Can you work these out from the model? Positions are in its coordinate system, mm. Round coordinates to 2 decimals unless told otherwise and drop trailing zeros. Loops run counter-clockwise (first coordinate to the right, second up) from the corner with the lowest first, then second, coordinate; pieces in that order, holes last.
(1) I want a section at A-A on y = 130. Write out the boundary of the cut face in (x, z).
(2) Will these pins go through, and if not, where does the flat tip stop? pin 1 Ø5 at (y, z) = (180.5, -30) entering from -X; pin 2 Ø25 at (y, z) = (527, 10) entering from -X; pin 3 Ø6 at (y, z) = (816, 2.5) entering from +X; pin 4 Ø22.5 at (y, z) = (50, -0.08) entering from -X.
(3) I want a section at C-C on y = 481.5. Write out the boundary of the cut face in (x, z).
(4) If I drill on line 1 along Z through (x, y) = (3, 1070); line 2 along Z through (x, y) = (15, 241); line 3 along Y through (x, z) = (-6, 7.5), over which ranges is the centre line in solid material (lowest first)?
(5) I want a section at B-B on z = -2.5. Write out the boundary of the cut face in (x, y), plus the area to 3 significant figures.
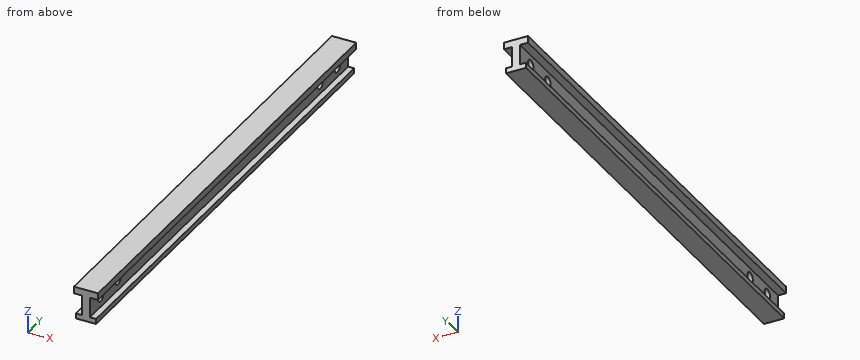
from build123d import *

# Parameters (mm, degrees)
BOSS_EXTRUDE1_DEPTH = 1200
CUT_EXTRUDE1_REACH  = 1203.333
SKETCH2_R           = 12.5


with BuildPart() as part:
    # Sketch1 → Boss-Extrude1 (new body)
    with BuildSketch(Plane(origin=(0, 0, 0), x_dir=(1, 0, 0), z_dir=(0, 1, 0))):
        Polygon((10, 27), (25, 27), (25, 40), (-25, 40), (-25, 27), (-10, 27), (-10, -23), (-30, -23), (-30, -40), (30, -40), (30, -23), (10, -23), align=None)
    extrude(amount=BOSS_EXTRUDE1_DEPTH)

    # Sketch2 → Cut-Extrude1 (cut, up to next)
    with BuildSketch(Plane(origin=(10, 0, 0), x_dir=(0, 0, -1), z_dir=(1, 0, 0)), mode=Mode.PRIVATE) as cut_extrude1_sk1:
        with Locations((1.916666667, 1150)):
            Circle(SKETCH2_R)
    cut_extrude1_tool1 = extrude(cut_extrude1_sk1.sketch, amount=-CUT_EXTRUDE1_REACH, mode=Mode.PRIVATE) & part.part
    # Sketch2 → Cut-Extrude1 (cut, up to next)
    with BuildSketch(Plane(origin=(10, 0, 0), x_dir=(0, 0, -1), z_dir=(1, 0, 0)), mode=Mode.PRIVATE) as cut_extrude1_sk2:
        with Locations((1.783333333, 1070)):
            Circle(SKETCH2_R)
    cut_extrude1_tool2 = extrude(cut_extrude1_sk2.sketch, amount=-CUT_EXTRUDE1_REACH, mode=Mode.PRIVATE) & part.part
    # Sketch2 → Cut-Extrude1 (cut, up to next)
    with BuildSketch(Plane(origin=(10, 0, 0), x_dir=(0, 0, -1), z_dir=(1, 0, 0)), mode=Mode.PRIVATE) as cut_extrude1_sk3:
        with Locations((0.083333333, 50)):
            Circle(SKETCH2_R)
    cut_extrude1_tool3 = extrude(cut_extrude1_sk3.sketch, amount=-CUT_EXTRUDE1_REACH, mode=Mode.PRIVATE) & part.part
    # Sketch2 → Cut-Extrude1 (cut, up to next)
    with BuildSketch(Plane(origin=(10, 0, 0), x_dir=(0, 0, -1), z_dir=(1, 0, 0)), mode=Mode.PRIVATE) as cut_extrude1_sk4:
        with Locations((0.216666667, 130)):
            Circle(SKETCH2_R)
    cut_extrude1_tool4 = extrude(cut_extrude1_sk4.sketch, amount=-CUT_EXTRUDE1_REACH, mode=Mode.PRIVATE) & part.part
    add(cut_extrude1_tool1.solids().sort_by_distance((10, 1150, -1.916667))[0], mode=Mode.SUBTRACT)
    add(cut_extrude1_tool2.solids().sort_by_distance((10, 1070, -1.783333))[0], mode=Mode.SUBTRACT)
    add(cut_extrude1_tool3.solids().sort_by_distance((10, 50, -0.083333))[0], mode=Mode.SUBTRACT)
    add(cut_extrude1_tool4.solids().sort_by_distance((10, 130, -0.216667))[0], mode=Mode.SUBTRACT)


solid = part.part
Filled sheet:
1. outline: (-30, 23) - (-10, 23) - (-10, 12.28) - (10, 12.28) - (10, 23) - (30, 23) - (30, 40) - (-30, 40) - close; (-25, -40) - (25, -40) - (25, -27) - (10, -27) - (10, -12.72) - (-10, -12.72) - (-10, -27) - (-25, -27) - close
2. pin 1: stops at x = -25
2. pin 2: stops at x = -10
2. pin 3: stops at x = 10
2. pin 4: passes through
3. outline: (-30, 23) - (-10, 23) - (-10, -27) - (-25, -27) - (-25, -40) - (25, -40) - (25, -27) - (10, -27) - (10, 23) - (30, 23) - (30, 40) - (-30, 40) - close
4. line 1: z = -40 to -14.28, 10.72 to 40
4. line 2: z = -40 to -27, 23 to 40
4. line 3: y = 0 to 40.06, 59.94 to 120.17, 139.83 to 1061.63, 1078.37 to 1141.78, 1158.22 to 1200
5. outline: (-10, 0) - (10, 0) - (10, 37.74) - (-10, 37.74) - close; (-10, 62.26) - (10, 62.26) - (10, 117.71) - (-10, 117.71) - close; (-10, 142.29) - (10, 142.29) - (10, 1057.52) - (-10, 1057.52) - close; (-10, 1082.48) - (10, 1082.48) - (10, 1137.51) - (-10, 1137.51) - close; (-10, 1162.49) - (10, 1162.49) - (10, 1200) - (-10, 1200) - close
5. area: 22,000 mm2
